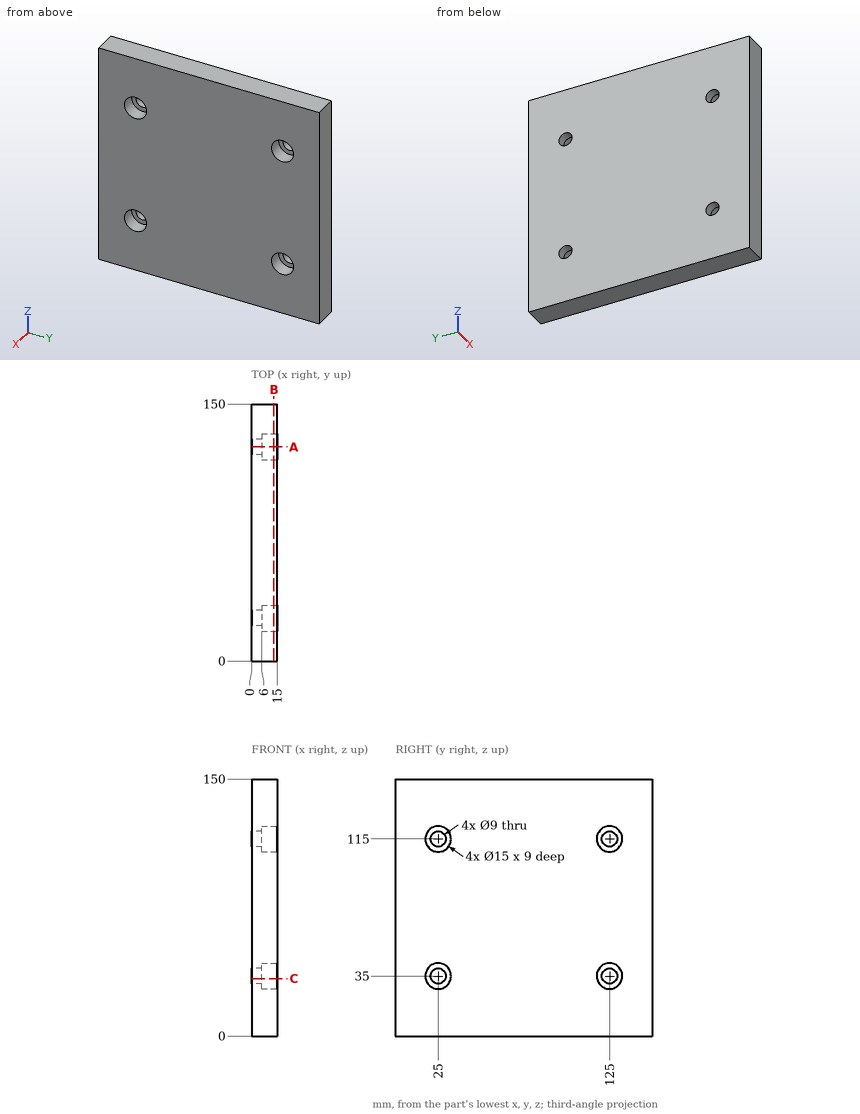
Print and shaded views of the part. All mm, measured from the part's lowest x, y and z. Round coordinates to 2 decimals unless told otherwise and drop trailing zeros. Write each loop counter-clockwise with the first axis right and the second up, starting at its lowest first coordinate (ties: lowest second). Pieces come first, ordered by that corner, then holes. Notation, with made-up numbers: (19, 8.25) -> (32, 8.25) arc R27 cw to (32, 38.25) -> close; hole circle Ø7 at (-24.5, 18.5). An arc over 180 degrees is marked (long way). Answer in a Markdown table with one row per item. Add a question column.
Item 1: Saw through at A-A, the plane y = 125. Write the cut outline in (x, z), then the cut area to 3 significant figures.
Item 2: Saw through at C-C, the plane z = 33.5. Write the cut outline in (x, y).
Item 3: Drop flat-ended pins along their axis: pin 1 Ø5.5 at (y, z) = (125, 115) entering from +X; pin 2 Ø4.5 at (y, z) = (128.5, 112.5) entering from +X. Give the stop position or say it passes through.
Item 4: Saw through at B-B, the plane x = 13. Write the cut outline in (y, z), then the cut area to 3 significant figures.
Item 5: Drill centre lines: line 1 (Y direction, x = 4.5, z = 115); line 2 (Y direction, x = 11.25, z = 115). Where is each one in solid material? Low to high. Write a range as from..to.
Findings below:
| question | item | result |
|---|---|---|
| 1 | outline | (0, 0) -> (15, 0) -> (15, 27.5) -> (6, 27.5) -> (6, 30.5) -> (0, 30.5) -> close; (0, 39.5) -> (6, 39.5) -> (6, 42.5) -> (15, 42.5) -> (15, 107.5) -> (6, 107.5) -> (6, 110.5) -> (0, 110.5) -> close; (0, 119.5) -> (6, 119.5) -> (6, 122.5) -> (15, 122.5) -> (15, 150) -> (0, 150) -> close |
| 1 | area | 1,870 mm^2 |
| 2 | outline | (0, 0) -> (15, 0) -> (15, 17.65) -> (6, 17.65) -> (6, 20.76) -> (0, 20.76) -> close; (0, 29.24) -> (6, 29.24) -> (6, 32.35) -> (15, 32.35) -> (15, 117.65) -> (6, 117.65) -> (6, 120.76) -> (0, 120.76) -> close; (0, 129.24) -> (6, 129.24) -> (6, 132.35) -> (15, 132.35) -> (15, 150) -> (0, 150) -> close |
| 3 | pin 1 | passes through |
| 3 | pin 2 | stops at x = 6 |
| 4 | outline | (0, 0) -> (150, 0) -> (150, 150) -> (0, 150) -> close; hole circle Ø15 at (25, 35); hole circle Ø15 at (25, 115); hole circle Ø15 at (125, 35); hole circle Ø15 at (125, 115) |
| 4 | area | 21,800 mm^2 |
| 5 | line 1 | y = 0..20.5, 29.5..120.5, 129.5..150 |
| 5 | line 2 | y = 0..17.5, 32.5..117.5, 132.5..150 |
